from build123d import *

# Parameters (mm, degrees)
SKETCH1_W           = 166.35
SKETCH1_H           = 160
SKETCH1_R           = 10.325
BOSS_EXTRUDE1_DEPTH = 14


with BuildPart() as part:
    # Sketch1 → Boss-Extrude1 (new body)
    with BuildSketch(Plane.XY):
        Rectangle(SKETCH1_W, SKETCH1_H)
        with Locations((-35.423, 50.048)):
            Circle(SKETCH1_R, mode=Mode.SUBTRACT)
        with Locations((-35.455423125, -34.102)):
            Circle(SKETCH1_R, mode=Mode.SUBTRACT)
        with Locations((32.852, -34.102)):
            Circle(SKETCH1_R, mode=Mode.SUBTRACT)
    extrude(amount=BOSS_EXTRUDE1_DEPTH)


solid = part.part
The model under review builds one solid part; all positions refer to its coordinate system, in mm. Give positions to 0.01 mm unless a question says otherwise; leave off trailing zeros. Loops run counter-clockwise (first coordinate to the right, second up) from the corner with the lowest first, then second, coordinate; pieces in that order, holes last. Notation, with made-up numbers: (-10.5, 7.5) -> (19.5, 7.5) arc R16 ccw to (19.5, 21.5) -> close; hole circle Ø10 at (65.25, -26.5). An arc over 180 degrees is marked (long way). Answer as a JSON object with one key per item and string values. Group by question number.
Q1. Take a section at A-A (y = -30). Write out the cut boundary in (x, z) (3 decimals).
Q2. Take a section at C-C (z = 6.5). Write out the cut boundary in (x, y) (3 decimals).
Q3. Draft analysis for pull direction X (two halves, no side actions). For faces 1 (the cylindrical face through (-25.607, -31.001, 6.902)), 2 (the flat face through (83.175, -1, 7)), 3 (the flat face through (-83.175, -1, 7)), state which applies: pulls with the +X half, pulls with the -X half, needs draft (parallel to the pull), parting line crosses it, or undercut.
Q4. Wall thickness on line 1 along X through (y, z) = (-35, 11.25) (3 decimals); line 2 along X through (y, z) = (-34, 8.75) (1 decimal); line 3 along Y through (x, z) = (-38.5, 2.5): over which ranges is each line inside the solid? List them lowest first.
Q5. Insertion check: pin 1 (18.5 mm diameter, centred on x = -35.423, y = 50.048, fed in from -Z). The pin has a flat end and moves straight along its axis. Give the tip position at first contact, or say it passes through.
Q6. Take a section at B-B (x = -39). Write out the cut boundary in (y, z), plus the area to 3 significant figures.
Answer below:
{
 "1": {"outline": "(-83.175, 0) -> (-44.931, 0) -> (-44.931, 14) -> (-83.175, 14) -> close; (-25.98, 0) -> (23.377, 0) -> (23.377, 14) -> (-25.98, 14) -> close; (42.327, 0) -> (83.175, 0) -> (83.175, 14) -> (42.327, 14) -> close"},
 "2": {"outline": "(-83.175, -80) -> (83.175, -80) -> (83.175, 80) -> (-83.175, 80) -> close; hole circle Ø20.65 at (-35.455, -34.102); hole circle Ø20.65 at (-35.423, 50.048); hole circle Ø20.65 at (32.852, -34.102)"},
 "3": {"face 1": "undercut", "face 2": "pulls with the +X half", "face 3": "pulls with the -X half"},
 "4": {"line 1": "x = -83.175 to -45.741, -25.17 to 22.566, 43.138 to 83.175", "line 2": "x = -83.2 to -45.8, -25.1 to 22.5, 43.2 to 83.2", "line 3": "y = -80 to -43.97, -24.24 to 40.19, 59.9 to 80"},
 "5": {"pin 1": "passes through"},
 "6": {"outline": "(-80, 0) -> (-43.8, 0) -> (-43.8, 14) -> (-80, 14) -> close; (-24.4, 0) -> (40.36, 0) -> (40.36, 14) -> (-24.4, 14) -> close; (59.73, 0) -> (80, 0) -> (80, 14) -> (59.73, 14) -> close", "area": "1,700 mm2"}
}
